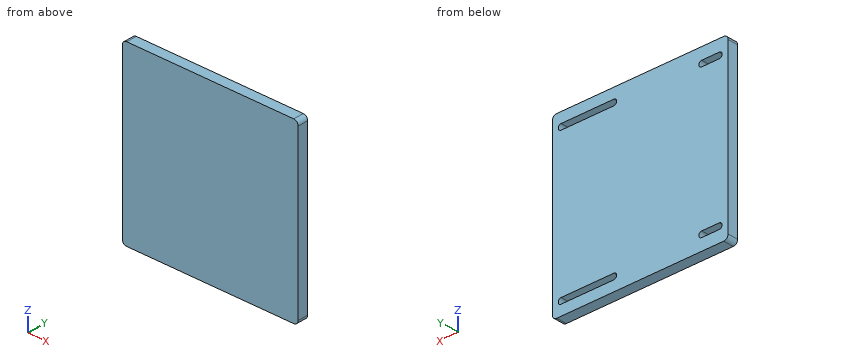
```python
from build123d import *

# Parameters (mm, degrees)
SKETCH_1_W          = 200
SKETCH_1_H          = 200
EXTRUDE_1_DEPTH     = 12
FILLET_1_R          = 5
CUT_EXTRUDE_1_DEPTH = 10


with BuildPart() as part:
    # 草图1 → 凸台-拉伸1 (new body)
    with BuildSketch(Plane(origin=(0, 0, 0), x_dir=(1, 0, 0), z_dir=(0, 1, 0))):
        Rectangle(SKETCH_1_W, SKETCH_1_H)
    extrude(amount=EXTRUDE_1_DEPTH)

    # 圆角1
    fillet_1_edges = [part.edges().sort_by_distance(p)[0] for p in [
        (100, 6, 100),
        (-100, 6, 100),
        (-100, 6, -100),
        (100, 6, -100),
    ]]
    fillet(fillet_1_edges, radius=FILLET_1_R)

    # 草图2 → 切除-拉伸1 (cut)
    with BuildSketch(Plane(origin=(0, 12, 0), x_dir=(1, 0, 0), z_dir=(0, 1, 0))):
        with BuildLine():
            Line((-90, 86.625), (-70, 86.625))
            ThreePointArc((-70, 86.625), (-66.75, 83.375), (-70, 80.125))
            Line((-70, 80.125), (-90, 80.125))
            ThreePointArc((-90, 80.125), (-93.25, 83.375), (-90, 86.625))
        make_face()
        with BuildLine():
            Line((-90, -86.625), (-70, -86.625))
            ThreePointArc((-70, -86.625), (-66.75, -83.375), (-70, -80.125))
            Line((-70, -80.125), (-90, -80.125))
            ThreePointArc((-90, -80.125), (-93.25, -83.375), (-90, -86.625))
        make_face()
        with BuildLine():
            Line((30, 88.25), (90, 88.25))
            ThreePointArc((90, 88.25), (93.25, 85), (90, 81.75))
            Line((90, 81.75), (30, 81.75))
            ThreePointArc((30, 81.75), (26.75, 85), (30, 88.25))
        make_face()
        with BuildLine():
            Line((30, -88.25), (90, -88.25))
            ThreePointArc((90, -88.25), (93.25, -85), (90, -81.75))
            Line((90, -81.75), (30, -81.75))
            ThreePointArc((30, -81.75), (26.75, -85), (30, -88.25))
        make_face()
    extrude(amount=-CUT_EXTRUDE_1_DEPTH, mode=Mode.SUBTRACT)


solid = part.part
```
Verification items for the finished model (mm, model axes). Coordinates: 2 decimals unless noted, no trailing zeros. Order: outer loops, then holes, each group sorted by start corner. A loop starts at its lowest first (then second) coordinate and runs counter-clockwise, first axis right, second up. Notation, with made-up numbers: (26.5, 45.5) - (75.5, 45.5) arc R20 ccw to (75.5, 60.5) - close; hole circle Ø10 at (-28, 75). An arc over 180 degrees is marked (long way). Return JSON: item names as keys, results as strings.
(1) Thickness scan on line 1 along Z through (x, y) = (-74, 10.75) (3 decimals); line 2 along Z through (x, y) = (38, 6.5); line 3 along X through (y, z) = (11.5, 82). Record the ranges inside material, lowest first.
Filled sheet:
{"line 1": "z = -100 to -86.625, -80.125 to 80.125, 86.625 to 100", "line 2": "z = -100 to -88.25, -81.75 to 81.75, 88.25 to 100", "line 3": "x = -100 to -92.94, -67.06 to 28.75, 91.25 to 100"}
(2) Section check A-A, the plane y = 8.75. Record the cut outline in (x, z) (3 decimals), and give its area (3 significant figures).
Filled sheet:
{"outline": "(-100, -95) arc R5 ccw to (-95, -100) - (95, -100) arc R5 ccw to (100, -95) - (100, 95) arc R5 ccw to (95, 100) - (-95, 100) arc R5 ccw to (-100, 95) - close; hole (-90, -86.625) - (-70, -86.625) arc R3.25 ccw to (-70, -80.125) - (-90, -80.125) arc R3.25 ccw to start; hole (-90, 80.125) - (-70, 80.125) arc R3.25 ccw to (-70, 86.625) - (-90, 86.625) arc R3.25 ccw to start; hole (30, -88.25) - (90, -88.25) arc R3.25 ccw to (90, -81.75) - (30, -81.75) arc R3.25 ccw to start; hole (30, 81.75) - (90, 81.75) arc R3.25 ccw to (90, 88.25) - (30, 88.25) arc R3.25 ccw to start", "area": "38,800 mm^2"}
(3) Go/stop test with a flat-tipped pin: pin 1 (2 mm diameter, centred on x = 52, z = -83.5, fed in from +Y). Record where the tip stops, or that it passes through.
Filled sheet:
{"pin 1": "stops at y = 2"}
(4) Section check B-B, the plane x = 47.5. Record the cut outline in (y, z), and give its area (3 significant figures).
Filled sheet:
{"outline": "(0, -100) - (12, -100) - (12, -88.25) - (2, -88.25) - (2, -81.75) - (12, -81.75) - (12, 81.75) - (2, 81.75) - (2, 88.25) - (12, 88.25) - (12, 100) - (0, 100) - close", "area": "2,270 mm^2"}
